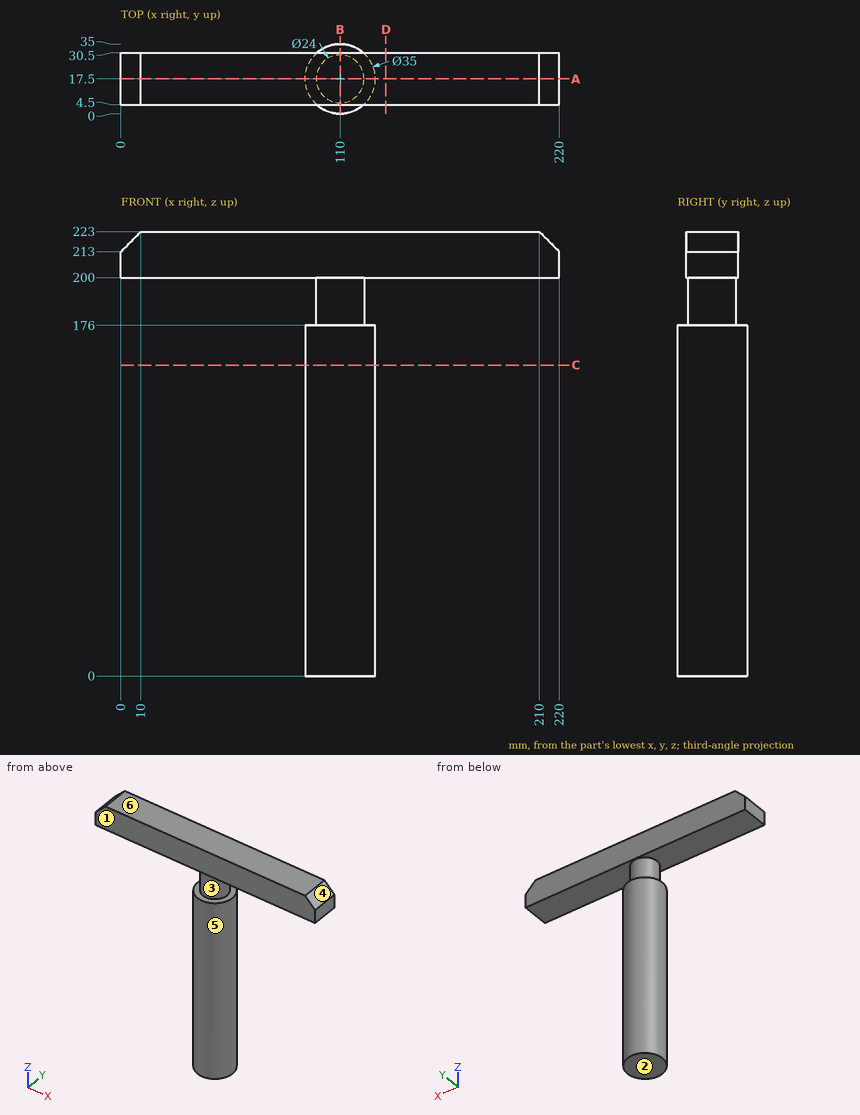
Geometry: see drawing. Coordinates: mm, zero at the bounding-box minimum. A direction names the side the tool comes from. Give positions to 0.01 mm unless a question says otherwise; leave off trailing zeros. Order: outer loops, then holes, each group sorted by start corner. A loop starts at its lowest first (then second) coordinate and runs counter-clockwise, first axis right, second up. Notation, with made-up numbers: M 43,2.25 L 51,2.25 A21 cw 51,31.25 Z; hole C -15.75,-23 d7. An arc over 180 degrees is marked long. Answer as CSV lines item,"result". Start each with the question number.
1) Cut plane B-B (x = 110). Output: boundary loops of the cut face in (y, z).
2) Mould query, pull axis Z, two halves, no side actions, for the marked faces 1, 2, 3 and 4. Classes: +Z half, -Z half, draft (parallel to the pull), parting line (faces both ways), or undercut.
3) Line query: line 1 (Z direction, x = 68, y = 12.5); line 2 (Y direction, x = 110, z = 134); line 3 (Y direction, x = 27, z = 204.5). Output: solid intervals per line, ascending. Write a range as from..to.
4) First-contact query: P1, Ø8, axis at x = 104.5, y = 18.5, coming from the -Z side; P2, Ø5, axis at y = 12.5, z = 196, coming from the +X side; P3, Ø2, axis at y = 18, z = 135, coming from the -X side; P4, Ø5, axis at x = 125.5, z = 128.5, coming from the -Y side. Flat tips, straight axial feed; report the tip coordinate or a pass-through.
5) Cut plane C-C (z = 156). Output: boundary loops of the cut face in (x, y).
6) Cut plane D-D (x = 133). Output: boundary loops of the cut face in (y, z).
7) Cut plane A-A (y = 17.5). Output: boundary loops of the cut face in (x, z).
8) Set-up query: the marked faces 5 and 6. Return all of +Z, -Z, +X, -X, +Y, -Y with unobstructed straight access to the full face (end or side cutting, diameter ignored); none if empty.
Findings below:
1,outline,"M 0,0 L 35,0 L 35,176 L 29.5,176 L 29.5,200 L 30.5,200 L 30.5,223 L 4.5,223 L 4.5,200 L 5.5,200 L 5.5,176 L 0,176 Z"
2,face 1,"draft"
2,face 2,"-Z half"
2,face 3,"undercut"
2,face 4,"+Z half"
3,line 1,"z = 200..223"
3,line 2,"y = 0..35"
3,line 3,"y = 4.5..30.5"
4,P1,"stops at z = 0"
4,P2,"stops at x = 121.74"
4,P3,"stops at x = 92.5"
4,P4,"stops at y = 5.78"
5,outline,"C 110,17.5 d35"
6,outline,"M 4.5,200 L 30.5,200 L 30.5,223 L 4.5,223 Z"
7,outline,"M 0,200 L 98,200 L 98,176 L 92.5,176 L 92.5,0 L 127.5,0 L 127.5,176 L 122,176 L 122,200 L 220,200 L 220,213 L 210,223 L 10,223 L 0,213 Z"
8,face 5,"-Z"
8,face 6,"+Z, +X, -X, +Y, -Y"
